Verification items for the finished model (mm, model axes). A direction names the side the tool comes from. Round coordinates to 2 decimals unless told otherwise and drop trailing zeros. Write each loop counter-clockwise with the first axis right and the second up, starting at its lowest first coordinate (ties: lowest second). Pieces come first, ordered by that corner, then holes. Notation, with made-up numbers: M 71.5,-21.5 L 97.5,-21.5 A12 ccw 97.5,-6.5 Z; hole C -1.5,-14 d10. An arc over 180 degrees is marked long. One line per item, written item: value. Start each with the question number.
Item 1: Tool access check on faces 1 (the face through (21, 0, 11)), 2 (the face through (-4, -4, 6)), 3 (the face through (12.45, 2.22, 1.29)), 4 (the face through (21, 0, 1)), 5 (the face through (0, -13, 6)). Record the directions out of +Z, -Z, +X, -X, +Y, -Y that give a thin tool (end or side, any length) a straight path to the whole face; none if there is none.
Item 2: Section check A-A, the plane x = -2.5. Record the cut outline in (y, z), then the cut area to 4 significant figures.
Item 3: Gauge pin test, flat ends, axial feed: pin 1 (12 mm diameter, centred on x = 2, y = 2.5, fed in from +Z); pin 2 (4 mm diameter, centred on x = -1.5, z = 5, fed in from +Y); pin 3 (2 mm diameter, centred on y = -11.5, z = 4.5, fed in from -X); pin 4 (1.5 mm diameter, centred on x = 25.5, z = 4.5, fed in from -Y). Record the tip position at first contact, or that the pin passes through.
Item 4: Section check C-C, the plane y = -4.5. Record the cut outline in (x, z).
Item 5: Section check B-B, the plane z = 10. Record the cut outline in (x, y).
Item 6: Thickness scan on probe 1 along X at (y, z) = (-5.45, 6.25); probe 2 along X at (y, z) = (-6, 5.5); probe 3 along X at (y, z) = (-16.25, 11.5). Record the ranges inside material, lowest first. Write a range as from..to.
Item 7: Section check D-D, the plane x = 19.5. Record the cut outline in (y, z).
from build123d import *

# Parameters (mm, degrees)
SERVO_CASE_WITH_MOUNTING_TABS_DEPTH = 12.5
TAB_MOUNTING_HOLE_SKETCH_R          = 1
TAB_MOUNTING_HOLE_DEPTH             = 2.5
OUTPUT_GEAR_BOSS_SKETCH_12_5_R      = 6.25
OUTPUT_GEAR_BOSS_12_5_DEPTH         = 4.5
OUTPUT_SHAFT_SKETCH_5_R             = 2.5
OUTPUT_SHAFT_5_DEPTH                = 3


with BuildPart() as part:
    # Servo Case Profile Sketch → Servo Case with Mounting Tabs (new body)
    with BuildSketch(Plane.XY):
        Polygon((0, 0), (0, -4), (-5, -4), (-5, -6.5), (0, -6.5), (0, -20), (22.5, -20), (22.5, -6.5), (27.5, -6.5), (27.5, -4), (22.5, -4), (22.5, 0), align=None)
    extrude(amount=SERVO_CASE_WITH_MOUNTING_TABS_DEPTH)

    # Tab Mounting Hole Sketch → Tab Mounting Hole (cut)
    with BuildSketch(Plane(origin=(0, -4, 0), x_dir=(1, 0, 0), z_dir=(0, 1, 0))):
        with Locations(Location((25, -6.25, 0), (0, 0, 270))):
            Circle(TAB_MOUNTING_HOLE_SKETCH_R)
        with Locations(Location((-2.5, -6.25, 0), (0, 0, 270))):
            Circle(TAB_MOUNTING_HOLE_SKETCH_R)
    extrude(amount=-TAB_MOUNTING_HOLE_DEPTH, mode=Mode.SUBTRACT)

    # Output Gear Boss Sketch Ø12.5 → Output Gear Boss Ø12.5 (add)
    with BuildSketch(Plane(origin=(0, 0, 0), x_dir=(1, 0, 0), z_dir=(0, 1, 0))):
        with Locations(Location((16.25, -6.25, 0), (0, 0, 270))):
            Circle(OUTPUT_GEAR_BOSS_SKETCH_12_5_R)
    extrude(amount=OUTPUT_GEAR_BOSS_12_5_DEPTH)

    # Output Shaft Sketch Ø5 → Output Shaft Ø5 (add)
    with BuildSketch(Plane(origin=(0, 4.5, 0), x_dir=(1, 0, 0), z_dir=(0, 1, 0))):
        with Locations(Location((16.25, -6.25, 0), (0, 0, 270))):
            Circle(OUTPUT_SHAFT_SKETCH_5_R)
    extrude(amount=OUTPUT_SHAFT_5_DEPTH)


solid = part.part
Response values:
1. face 1: +Z, +X, +Y
1. face 2: +Z, -Z, -X, +Y
1. face 3: +Y
1. face 4: -Z, +X, +Y
1. face 5: +Z, -Z, -X, -Y
2. outline: M -6.5,0 L -4,0 L -4,5.25 L -6.5,5.25 Z; M -6.5,7.25 L -4,7.25 L -4,12.5 L -6.5,12.5 Z
2. area: 26.25 mm2
3. pin 1: stops at z = 12.5
3. pin 2: stops at y = 0
3. pin 3: stops at x = 0
3. pin 4: stops at y = -6.5
4. outline: M -5,0 L 27.5,0 L 27.5,12.5 L -5,12.5 Z; hole C -2.5,6.25 d2; hole C 25,6.25 d2
5. outline: M -5,-6.5 L 0,-6.5 L 0,-20 L 22.5,-20 L 22.5,-6.5 L 27.5,-6.5 L 27.5,-4 L 22.5,-4 L 22.5,0 L 21.25,0 L 21.25,4.5 L 11.25,4.5 L 11.25,0 L 0,0 L 0,-4 L -5,-4 Z
6. probe 1: x = -5..-3.5, -1.5..24, 26..27.5
6. probe 2: x = -5..-3.16, -1.84..24.34, 25.66..27.5
6. probe 3: x = 0..22.5
7. outline: M -20,0 L 0,0 L 0,0.91 L 4.5,0.91 L 4.5,11.59 L 0,11.59 L 0,12.5 L -20,12.5 Z
